from build123d import *

# Parameters (mm, degrees)
BASE_BODY_DEPTH         = 12
BASE_BODY_2_DEPTH       = 12
FOOT_BOSS_60_DEPTH      = 60
WINDOW_CUT_DEPTH        = 60
SADDLE_ENDS_98_DEPTH    = 98
SADDLE_CRADLE_CUT_DEPTH = 19
ARCH_RELIEF_CUT_DEPTH   = 93
RETAINING_START         = 2
RETAINING_LIP_A_DEPTH   = 2
RETAINING_LIP_B_DEPTH   = 2


with BuildPart() as part:
    # Base Body Sketch → Base Body (new body)
    with BuildSketch(Plane(origin=(0, 0, 0), x_dir=(1, 0, 0), z_dir=(0, 1, 0))):
        with BuildLine():
            Line((-41, -14), (41, -14))
            ThreePointArc((41, -14), (49, -22), (41, -30))
            Line((41, -30), (-41, -30))
            ThreePointArc((-41, -30), (-49, -22), (-41, -14))
        make_face()
    extrude(amount=BASE_BODY_DEPTH)



with BuildPart() as body_2:
    # Base Body Sketch → Base Body 2 (new body)
    with BuildSketch(Plane(origin=(0, 0, 0), x_dir=(1, 0, 0), z_dir=(0, 1, 0))):
        with BuildLine():
            Line((41, 30), (-41, 30))
            ThreePointArc((-41, 30), (-49, 22), (-41, 14))
            Line((-41, 14), (41, 14))
            ThreePointArc((41, 14), (49, 22), (41, 30))
        make_face()
    extrude(amount=BASE_BODY_2_DEPTH)


with BuildPart() as part_1:
    add(part.part)

    add(body_2.part)  # Foot Boss 60 merges body 2
    # Foot Boss Sketch → Foot Boss 60 (add)
    with BuildSketch(Plane(origin=(30, 0, 0), x_dir=(0, 0, -1), z_dir=(1, 0, 0))):
        with BuildLine():
            Line((-14, 12), (-30, 12))
            Line((-30, 12), (-30, 56))
            Line((-30, 56), (30, 56))
            Line((30, 56), (30, 12))
            Line((30, 12), (14, 12))
            ThreePointArc((14, 12), (0, 26), (-14, 12))
        make_face()
    extrude(amount=-FOOT_BOSS_60_DEPTH)

    # Window Cut Sketch → Window Cut (cut)
    with BuildSketch(Plane(origin=(30, 0, 0), x_dir=(0, 0, -1), z_dir=(1, 0, 0))):
        Polygon((-23.08335547, 59.033182801), (-30, 12), (-33.835274918, 12), (-33.835274918, 59.033182801), align=None)
        Polygon((23.08335547, 59.033182801), (30, 12), (40.995792327, 12), (40.995792327, 59.033182801), align=None)
    extrude(amount=-WINDOW_CUT_DEPTH, mode=Mode.SUBTRACT)

    # Saddle Ends Sketch → Saddle Ends 98 (add)
    with BuildSketch(Plane(origin=(49, 0, 0), x_dir=(0, 0, -1), z_dir=(1, 0, 0))):
        with BuildLine():
            Line((10, 82), (20, 82))
            Line((20, 82), (23.529411765, 56))
            Line((23.529411765, 56), (-23.529411765, 56))
            Line((-23.529411765, 56), (-20, 82))
            Line((-20, 82), (-10, 82))
            ThreePointArc((-10, 82), (0, 72), (10, 82))
        make_face()
    extrude(amount=-SADDLE_ENDS_98_DEPTH)

    # Saddle Cradle Cut Sketch → Saddle Cradle Cut (cut)
    with BuildSketch(Plane(origin=(0, 82, 0), x_dir=(1, 0, 0), z_dir=(0, 1, 0))):
        Polygon((26, 0), (26, -36.490977082), (-26, -36.490977082), (-26, 35.721826881), (26, 35.721826881), align=None)
    extrude(amount=-SADDLE_CRADLE_CUT_DEPTH, mode=Mode.SUBTRACT)

    # Arch Relief Cut Sketch → Arch Relief Cut (cut)
    with BuildSketch(Plane(origin=(0, 0, -30), x_dir=(-1, 0, 0), z_dir=(0, 0, -1))):
        Polygon((0, 24), (12, 24), (12, 48), (-12, 48), (-12, 24), align=None)
    extrude(amount=-ARCH_RELIEF_CUT_DEPTH, mode=Mode.SUBTRACT)

    # Retaining Lip A Sketch → Retaining Lip A (add)
    with BuildSketch(Plane(origin=(49, 0, 0), x_dir=(0, 0, -1), z_dir=(1, 0, 0)).offset(RETAINING_START)):
        with BuildLine():
            Line((-12, 82), (-10, 82))
            ThreePointArc((-10, 82), (0, 72), (10, 82))
            Line((10, 82), (12, 82))
            ThreePointArc((12, 82), (0, 70), (-12, 82))
        make_face()
    extrude(amount=-RETAINING_LIP_A_DEPTH)

    # Retaining Lip B Sketch → Retaining Lip B (add)
    with BuildSketch(Plane.ZY.offset(49)):
        with BuildLine():
            Line((10, 82), (12, 82))
            ThreePointArc((12, 82), (0, 70), (-12, 82))
            Line((-12, 82), (-10, 82))
            ThreePointArc((-10, 82), (0, 72), (10, 82))
        make_face()
    extrude(amount=RETAINING_LIP_B_DEPTH)


solid = part_1.part
Model file for the job. Use its own axes, mm. A direction names the side the tool comes from. Give positions to 0.01 mm unless a question says otherwise; leave off trailing zeros. Loops run counter-clockwise (first coordinate to the right, second up) from the corner with the lowest first, then second, coordinate; pieces in that order, holes last.
1) Tool access for faces 5 (the flat face through (12, 36, 0)), 6 (the flat face through (30, 34, 0)), 7 (the flat face through (0, 63, 0)): list every direction of +Z, -Z, +X, -X, +Y, -Y with a clear straight run to the whole face (end or side of a thin tool).
2) Saw through at B-B (y = 7). Write the cut outline in (x, z).
3) Wall check: line 1 (X direction, y = 27, z = -13.5); line 2 (Y direction, x = 38.5, z = 15.5); line 3 (Z direction, x = 7, y = 11.5). Give the ranges that are in metal, low to high.
4) Saw through at D-D (x = 22.5). Write the cut outline in (y, z), plus the area to 3 significant figures.
5) Saw through at C-C (z = 8.5). Write the cut outline in (x, y), plus the area to 3 significant figures.
6) Saw through at A-A (x = -37). Write the cut outline in (y, z).
7) Pull direction Y, two halves, no side cores. Call faces 1 (the cylindrical face through (-49, 6, 22)), 2 (the flat face through (0, 24, -18)), 3 (the flat face through (13.75, 34.31, -26.72)), 4 (the flat face through (-12, 36, 0)): +Y half, -Y half, draft (parallel to the pull), parting line (faces both ways), or undercut.
8) Flat gauge pins, fed straight in: pin 1 Ø22 at (y, z) = (37, 2.5) entering from +X; pin 2 Ø9.5 at (y, z) = (70.5, -4.5) entering from +X; pin 3 Ø5.5 at (y, z) = (68, 7) entering from -X; pin 4 Ø12 at (y, z) = (39, 8) entering from -X. Where does each tip first touch, or does it go through?
Answer block:
1. face 5: +Z, -Z
1. face 6: +Z, -Z, +X
1. face 7: +Z, -Z, +Y
2. outline: (-41, -30) - (41, -30) arc R8 ccw to (41, -14) - (-41, -14) arc R8 ccw to start; (-41, 14) - (41, 14) arc R8 ccw to (41, 30) - (-41, 30) arc R8 ccw to start
3. line 1: x = -30 to -12, 12 to 30
3. line 2: y = 0 to 12, 56 to 82
3. line 3: z = -30 to -14, 14 to 30
4. outline: (0, -30) - (12, -30) - (56, -23.53) - (63, -22.58) - (63, 22.58) - (56, 23.53) - (12, 30) - (0, 30) - (0, 14) - (12, 14) arc R14 cw to (12, -14) - (0, -14) - close
4. area: 2,750 mm2
5. outline: (-51, 73.53) - (-49, 73.53) - (-49, 56) - (-30, 56) - (-30, 23.12) - (30, 23.12) - (30, 56) - (49, 56) - (49, 73.53) - (51, 73.53) - (51, 76.73) - (26, 76.73) - (26, 63) - (-26, 63) - (-26, 76.73) - (-51, 76.73) - close; hole (-12, 24) - (12, 24) - (12, 48) - (-12, 48) - close
5. area: 2,730 mm2
6. outline: (0, -30) - (12, -30) - (12, -14) - (0, -14) - close; (0, 14) - (12, 14) - (12, 30) - (0, 30) - close; (56, -23.53) - (82, -20) - (82, -10) arc R10 cw to (82, 10) - (82, 20) - (56, 23.53) - close
7. face 1: draft
7. face 2: undercut
7. face 3: +Y half
7. face 4: undercut
8. pin 1: stops at x = 30
8. pin 2: stops at x = 51
8. pin 3: stops at x = -49
8. pin 4: stops at x = -30
